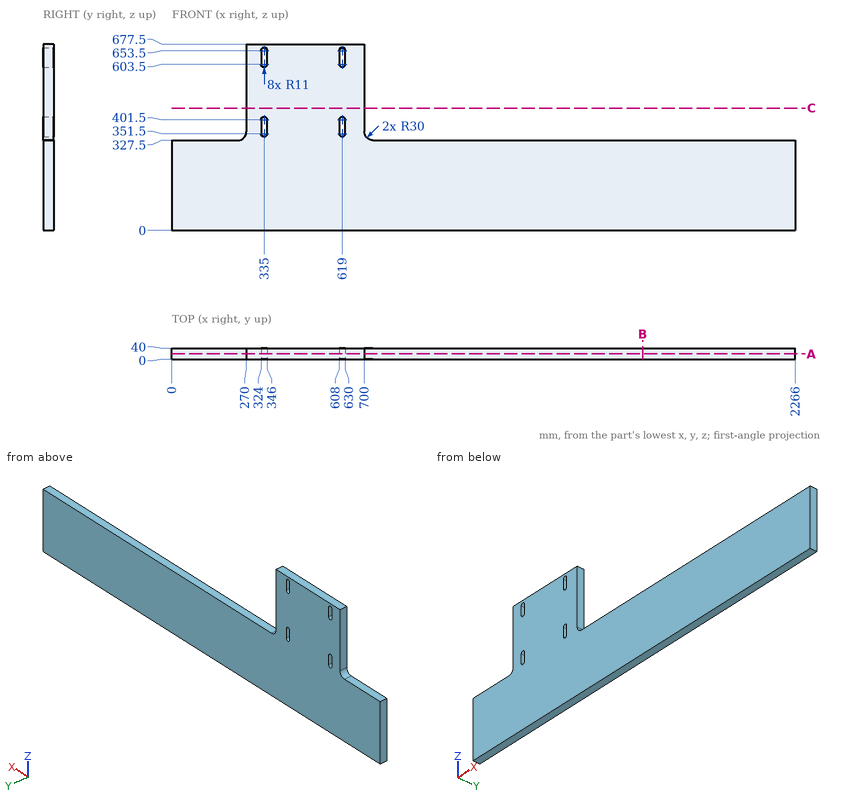
For this review, use the dimensioned drawing (mm, ordinates from the lowest corner) and the shaded views. Give positions to 0.01 mm unless a question says otherwise; leave off trailing zeros. Write each loop counter-clockwise with the first axis right and the second up, starting at its lowest first coordinate (ties: lowest second). Pieces come first, ordered by that corner, then holes. Notation, with made-up numbers: M 87,-6.75 L 115,-6.75 A18 cw 115,24.25 Z; hole C 80.5,-32 d1. An arc over 180 degrees is marked long. Answer as a JSON object with one key per item and string values. Group by question number.
Item 1: For probe 1 along X at (y, z) = (26, 353); probe 2 along Z at (x, y) = (1598, 33); probe 3 along X at (y, z) = (35, 595), list the stretches that pass through material, from the lowest coordinate up. Write a range as [from, to].
Item 2: Consider section C-C on z = 444. Write out the cut boundary in (x, y).
Item 3: For pin 1 Ø1 at (y, z) = (16, 386) entering from -X; pin 2 Ø6 at (y, z) = (31, 438.5) entering from +X; pin 3 Ø20 at (x, y) = (81, 10) entering from +Z, all flat-tipped, find the tip position at first contact; note any pin that passes through.
Item 4: Consider section A-A on y = 20. Write out the cut boundary in (x, z).
Item 5: Consider section B-B on x = 1712. Write out the cut boundary in (y, z).
Check result:
{
 "1": {"probe 1": "x = [269.66, 324], [346, 608], [630, 700.34]", "probe 2": "z = [0, 327.5]", "probe 3": "x = [270, 328.02], [341.98, 612.02], [625.98, 700]"},
 "2": {"outline": "M 270,0 L 700,0 L 700,40 L 270,40 Z"},
 "3": {"pin 1": "stops at x = 270", "pin 2": "stops at x = 700", "pin 3": "stops at z = 327.5"},
 "4": {"outline": "M 0,0 L 2266,0 L 2266,327.5 L 730,327.5 A30 cw 700,357.5 L 700,677.5 L 270,677.5 L 270,357.5 A30 cw 240,327.5 L 0,327.5 Z; hole M 324,351.5 A11 ccw 346,351.5 L 346,401.5 A11 ccw 324,401.5 Z; hole M 324,603.5 A11 ccw 346,603.5 L 346,653.5 A11 ccw 324,653.5 Z; hole M 608,351.5 A11 ccw 630,351.5 L 630,401.5 A11 ccw 608,401.5 Z; hole M 608,603.5 A11 ccw 630,603.5 L 630,653.5 A11 ccw 608,653.5 Z"},
 "5": {"outline": "M 0,0 L 40,0 L 40,327.5 L 0,327.5 Z"}
}
